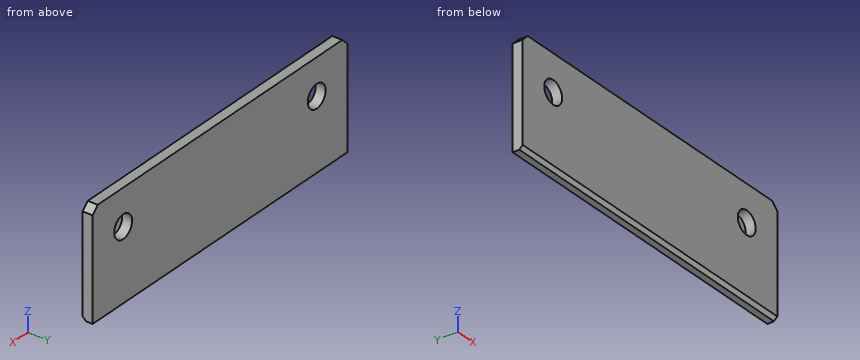
```python
from build123d import *

# Parameters (mm, degrees)
SKETCH1_W           = 50
SKETCH1_H           = 16.3
BOSS_EXTRUDE1_DEPTH = 1.5
SKETCH3_R           = 1.75
CUT_EXTRUDE2_DEPTH  = 10
CHAMFER1_SIZE       = 1
CHAMFER2_SIZE       = 0.5


with BuildPart() as part:
    # Sketch1 → Boss-Extrude1 (new body)
    with BuildSketch(Plane(origin=(0, 0, 0), x_dir=(1, 0, 0), z_dir=(0, 1, 0))):
        Rectangle(SKETCH1_W, SKETCH1_H)
    extrude(amount=BOSS_EXTRUDE1_DEPTH)

    # Sketch3 → Cut-Extrude2 (cut)
    with BuildSketch(Plane(origin=(0, 1.5, 0), x_dir=(1, 0, 0), z_dir=(0, 1, 0))):
        with Locations(Location((-19, -2.65, 0), (0, 0, 270))):
            Circle(SKETCH3_R)
        with Locations(Location((19, -2.65, 0), (0, 0, 270))):
            Circle(SKETCH3_R)
    extrude(amount=-CUT_EXTRUDE2_DEPTH, mode=Mode.SUBTRACT)

    # Chamfer1
    chamfer1_edges = [part.edges().sort_by_distance(p)[0] for p in [
        (25, 0.75, 8.15),
        (-25, 0.75, 8.15),
    ]]
    chamfer(chamfer1_edges, length=CHAMFER1_SIZE)

    # Chamfer2
    chamfer2_edges = [part.edges().sort_by_distance(p)[0] for p in [
        (0, 0, -8.15),
    ]]
    chamfer(chamfer2_edges, length=CHAMFER2_SIZE)


solid = part.part
```
Check sheet for the modelled part. Datum: model origin and axes. Units: mm. Coordinates: 2 decimals unless noted, no trailing zeros. Write each loop counter-clockwise with the first axis right and the second up, starting at its lowest first coordinate (ties: lowest second). Pieces come first, ordered by that corner, then holes. Notation, with made-up numbers: (-28, -11) -> (-5, -11) arc R18 ccw to (-5, 14) -> close; hole circle Ø7 at (31.5, 68). An arc over 180 degrees is marked (long way). Use a Markdown table: item, result.
1. Scan lines: line 1 along X through (y, z) = (1.15, 2.65); line 2 along X through (y, z) = (0.2, 3.5); line 3 along Z through (x, y) = (-17.5, 0.7). Record each from-to range of solid material in increasing order.
Reported:
| item | result |
|---|---|
| line 1 | x = -25 to -20.75, -17.25 to 17.25, 20.75 to 25 |
| line 2 | x = -25 to -20.53, -17.47 to 17.47, 20.53 to 25 |
| line 3 | z = -8.15 to 1.75, 3.55 to 8.15 |
2. Sectioned sample at A-A (y = 0.9). Enter the section's corners in (x, z), plus the area to 3 significant figures.
Reported:
| item | result |
|---|---|
| outline | (-25, -8.15) -> (25, -8.15) -> (25, 7.15) -> (24, 8.15) -> (-24, 8.15) -> (-25, 7.15) -> close; hole circle Ø3.5 at (-19, 2.65); hole circle Ø3.5 at (19, 2.65) |
| area | 795 mm2 |
3. Sectioned sample at B-B (z = 2.65). Enter the section's corners in (x, y), plus the area to 3 significant figures.
Reported:
| item | result |
|---|---|
| outline | (-25, 0) -> (-20.75, 0) -> (-20.75, 1.5) -> (-25, 1.5) -> close; (-17.25, 0) -> (17.25, 0) -> (17.25, 1.5) -> (-17.25, 1.5) -> close; (20.75, 0) -> (25, 0) -> (25, 1.5) -> (20.75, 1.5) -> close |
| area | 64.5 mm2 |
4. Sectioned sample at C-C (x = 19). Enter the section's corners in (y, z), plus the area to 3 significant figures.
Reported:
| item | result |
|---|---|
| outline | (0, -7.65) -> (0.5, -8.15) -> (1.5, -8.15) -> (1.5, 0.9) -> (0, 0.9) -> close; (0, 4.4) -> (1.5, 4.4) -> (1.5, 8.15) -> (0, 8.15) -> close |
| area | 19.1 mm2 |
5. Go/stop test with a flat-tipped pin: pin 1 Ø3 at (x, z) = (19, 2.65) entering from +Y. Record where the tip stops, or that it passes through.
Reported:
| item | result |
|---|---|
| pin 1 | passes through |
